Could you check a few things on this drawing? It's one solid part, dimensions in mm from its lowest x, y, z. Give positions to 0.01 mm unless a question says otherwise; leave off trailing zeros. Loops run counter-clockwise (first coordinate to the right, second up) from the corner with the lowest first, then second, coordinate; pieces in that order, holes last. Notation, with made-up numbers: (-13.75, 20.25) - (15.25, 20.25) arc R22 cw to (15.25, 27.25) - close; hole circle Ø10 at (-36, -18). An arc over 180 degrees is marked (long way). Return JSON: item names as keys, results as strings. Group by question number.
(1) For P1, Ø2, axis at y = 36.5, z = 11, coming from the -X side, with a flat end and sliding along its axis, tell me the tip position at first contact or that it passes through.
(2) If we section it at D-D (y = 241): Please give me the cut outline in (x, z), then the cut area to 3 significant figures.
(3) If we section it at B-B (x = 30): Please give me the cut outline in (y, z), then the cut area to 3 significant figures.
(4) If we mould it in two halves opening along Y, with no side actions, what happens to the marked faces 1, 2, 3 and 4? For each: released by +Y, released by -Y, zero draft, split by the parting line, or undercut.
(5) If we section it at C-C (z = 17.75): Please give me the cut outline in (x, y).
(6) If we section it at A-A (y = 128): Please give me the cut outline in (x, z), then the cut area to 3 significant figures.
(7) I need wall thicknesses on probe 1 along Y at (x, z) = (30, 16); probe 2 along X at (y, z) = (128, 9); probe 3 along Y at (x, z) = (31.5, 2.5). Which ranges of each line are inside material? Lowest first, please. Write a range as [from, to].
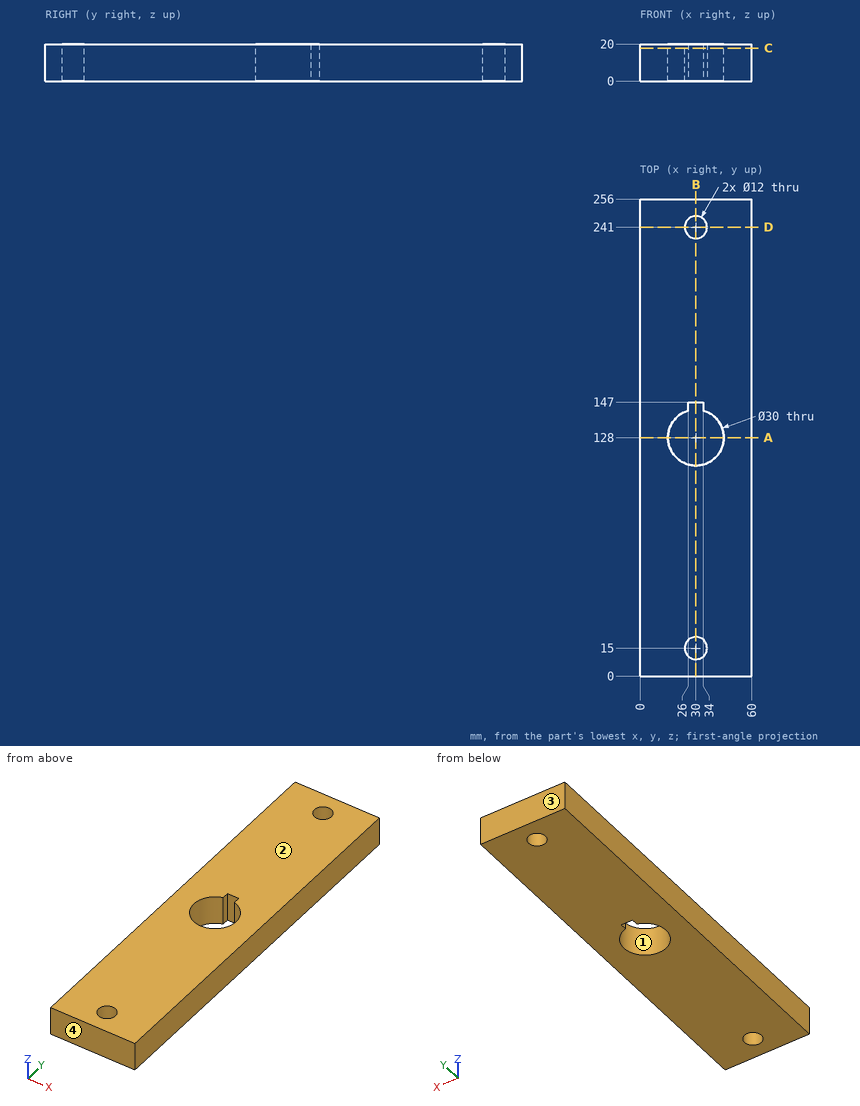
Values:
{
 "1": {"P1": "x = 0"},
 "2": {"outline": "(0, 0) - (24, 0) - (24, 20) - (0, 20) - close; (36, 0) - (60, 0) - (60, 20) - (36, 20) - close", "area": "960 mm2"},
 "3": {"outline": "(0, 0) - (9, 0) - (9, 20) - (0, 20) - close; (21, 0) - (113, 0) - (113, 20) - (21, 20) - close; (147, 0) - (235, 0) - (235, 20) - (147, 20) - close; (247, 0) - (256, 0) - (256, 20) - (247, 20) - close", "area": "3,960 mm2"},
 "4": {"face 1": "undercut", "face 2": "zero draft", "face 3": "released by +Y", "face 4": "released by -Y"},
 "5": {"outline": "(0, 0) - (60, 0) - (60, 256) - (0, 256) - close; hole circle Ø12 at (30, 15); hole circle Ø12 at (30, 241); hole (26, 142.46) arc R15 ccw (long way) to (34, 142.46) - (34, 147) - (26, 147) - close"},
 "6": {"outline": "(0, 0) - (15, 0) - (15, 20) - (0, 20) - close; (45, 0) - (60, 0) - (60, 20) - (45, 20) - close", "area": "600 mm2"},
 "7": {"probe 1": "[0, 9], [21, 113], [147, 235], [247, 256]", "probe 2": "[0, 15], [45, 60]", "probe 3": "[0, 9.19], [20.81, 113.08], [147, 235.19], [246.81, 256]"}
}
